```python
from build123d import *

# Parameters (mm, degrees)
EXTRUDE_1_DEPTH               = 10
EXTRUDE_2_DEPTH               = 5
EXTRUDE_2_DEPTH_BACK          = 5
EXTRUDE_2_START               = -2.5
CUT_EXTRUDE_3_DEPTH           = 308.667661103
CUT_EXTRUDE_3_DEPTH_BACK      = 308.667661103
SKETCH_4_W                    = 20
SKETCH_4_H                    = 2.700809371
CUT_EXTRUDE_2_DEPTH           = 308.667661103
CUT_EXTRUDE_2_DEPTH_BACK      = 308.667661103
SKETCH_5_W                    = 1
SKETCH_5_H                    = 14.903200109
SKETCH_8_W                    = 10
SKETCH_8_H                    = 1.5
EXTRUDE_2_2_DEPTH             = 10
EXTRUDE_2_2_DIRECTION_2_REACH = 314.682
SKETCH_11_W                   = 20
SKETCH_11_H                   = 26.003490823
CUT_EXTRUDE_4_DEPTH           = 10
EXTRUDE_3_DEPTH               = 15
CUT_EXTRUDE_5_DEPTH           = 318.837559332
CUT_EXTRUDE_5_DEPTH_BACK      = 318.837559332
SKETCH_13_R                   = 3
EXTRUDE_4_DEPTH               = 50


with BuildPart() as part:
    # 草图1 → 凸台-拉伸1 (new, symmetric)
    with BuildSketch(Plane.XY):
        Polygon((0, 0), (138.199336083, 164.699555271), (145.269999789, 173.126044145), (149.100222005, 169.912106096), (142.029558298, 161.485617222), (10.722534603, 5), (4.294658506, -2.660444431), (30, -2.660444431), (30, -7.660444431), (-6.427876097, -7.660444431), align=None)
    extrude(amount=EXTRUDE_1_DEPTH, both=True)

    # 草图3 → Extrude 2 (add, two sides: drawn at the far end of the back side and taken through both)
    with BuildSketch(Plane(origin=(0, 0, 0), x_dir=(0, 0, 1), z_dir=(-0.766044443118979, 0.642787609686538, 0)).offset(EXTRUDE_2_START - EXTRUDE_2_DEPTH_BACK)):
        with BuildLine():
            Line((-17.5, 226.389937847), (-17.5, 226.243201682))
            Line((-17.5, 226.243201682), (-17.5, 222.5))
            Line((-17.5, 222.5), (-7.5, 222.5))
            Line((-7.5, 222.5), (-7.5, 223.5))
            Line((-7.5, 223.5), (7.5, 223.5))
            Line((7.5, 223.5), (7.5, 222.5))
            Line((7.5, 222.5), (17.5, 222.5))
            Line((17.5, 222.5), (17.5, 226.243201682))
            Line((17.5, 226.243201682), (17.5, 226.389937847))
            ThreePointArc((17.5, 226.389937847), (0, 300.243201682), (-17.5, 226.389937847))
        make_face()
        with BuildLine():
            Line((-15, 227.967835418), (-15, 226.243201682))
            Line((-15, 226.243201682), (-15, 225))
            Line((-15, 225), (-10, 225))
            Line((-10, 225), (-10, 226))
            Line((-10, 226), (10, 226))
            Line((10, 226), (10, 225))
            Line((10, 225), (15, 225))
            Line((15, 225), (15, 226.243201682))
            Line((15, 226.243201682), (15, 227.967835418))
            ThreePointArc((15, 227.967835418), (0, 297.743201682), (-15, 227.967835418))
        make_face(mode=Mode.SUBTRACT)
    extrude(amount=EXTRUDE_2_DEPTH + EXTRUDE_2_DEPTH_BACK)

    # 草图4 → 切除-拉伸3 (cut, two sides: drawn at the far end of the back side and taken through both)
    with BuildSketch(Plane(origin=(0, 0, 0), x_dir=(0, 0, 1), z_dir=(-0.7660444431189785, 0.6427876096865388, 0)).offset(-CUT_EXTRUDE_3_DEPTH_BACK)):
        with Locations((0, 226.350404685)):
            Rectangle(SKETCH_4_W, SKETCH_4_H)
    extrude(amount=CUT_EXTRUDE_3_DEPTH + CUT_EXTRUDE_3_DEPTH_BACK, mode=Mode.SUBTRACT)

    # 草图5 → 切除-拉伸2 (cut, two sides: drawn at the far end of the back side and taken through both)
    with BuildSketch(Plane(origin=(0, 0, 0), x_dir=(0, 0, 1), z_dir=(-0.7660444431189785, 0.6427876096865388, 0)).offset(-CUT_EXTRUDE_2_DEPTH_BACK)):
        with Locations((0, 297.743201683)):
            Rectangle(SKETCH_5_W, SKETCH_5_H)
    extrude(amount=CUT_EXTRUDE_2_DEPTH + CUT_EXTRUDE_2_DEPTH_BACK, mode=Mode.SUBTRACT)

    # 草图8 → Extrude 2 2 (add)
    with BuildSketch(Plane(origin=(192.990549633, 229.997180861, 0), x_dir=(0.766044443118979, -0.6427876096865381, 0), z_dir=(0.6427876096865381, 0.766044443118979, 0))):
        with Locations((2.5, -1.25)):
            Rectangle(SKETCH_8_W, SKETCH_8_H)
    extrude_2_2 = extrude(amount=EXTRUDE_2_2_DEPTH)

    # 草图8 → Extrude 2 2 direction 2 (add, up to next)
    with BuildSketch(Plane(origin=(192.990549633, 229.997180861, 0), x_dir=(0.766044443118979, -0.6427876096865381, 0), z_dir=(0.6427876096865381, 0.766044443118979, 0)), mode=Mode.PRIVATE) as extrude_2_2_direction_2_sk1:
        with Locations((2.5, -1.25)):
            Rectangle(SKETCH_8_W, SKETCH_8_H)
    extrude_2_2_direction_2_tool1 = extrude(extrude_2_2_direction_2_sk1.sketch, amount=-EXTRUDE_2_2_DIRECTION_2_REACH, mode=Mode.PRIVATE) - part.part
    extrude_2_2_direction_2 = extrude_2_2_direction_2_tool1.solids().sort_by_distance((194.905661, 228.390212, 1.25))[0]
    add(extrude_2_2_direction_2)

    # 镜向1: Extrude 2 2, Extrude 2 2 direction 2 across plane
    add(extrude_2_2.mirror(Plane.XY))
    add(extrude_2_2_direction_2.mirror(Plane.XY))

    # 草图11 → 切除-拉伸4 (cut)
    with BuildSketch(Plane.XZ.offset(7.660444431)):
        with Locations((20, -3.001745411)):
            Rectangle(SKETCH_11_W, SKETCH_11_H)
    extrude(amount=-CUT_EXTRUDE_4_DEPTH, mode=Mode.SUBTRACT)

    # 草图12 → 凸台-拉伸3 (add)
    with BuildSketch(Plane.XY.offset(10)):
        Polygon((4.294658506, -2.660444431), (-2.232377941, -2.660444431), (-6.427876097, -7.660444431), (10, -7.660444431), (10, -2.660444431), align=None)
    extrude_3 = extrude(amount=EXTRUDE_3_DEPTH)

    # 镜向2: 凸台-拉伸3 across plane
    add(extrude_3.mirror(Plane.XY))

    # 草图13 → 切除-拉伸5 (cut, two sides: drawn at the far end of the back side and taken through both)
    with BuildSketch(Plane(origin=(0, 0, -2), x_dir=(-1, 0, 0), z_dir=(0, 0, -1)).offset(-CUT_EXTRUDE_5_DEPTH_BACK)):
        with Locations((-198.163787282, 232.207589437)):
            Circle(SKETCH_13_R)
    extrude(amount=CUT_EXTRUDE_5_DEPTH + CUT_EXTRUDE_5_DEPTH_BACK, mode=Mode.SUBTRACT)

    # 草图14 → 凸台-拉伸4 (add)
    with BuildSketch(Plane(origin=(0, 0, -25), x_dir=(-1, 0, 0), z_dir=(0, 0, -1))):
        Polygon((2.232377941, -2.660444431), (6.427876097, -2.660444431), (14.127876097, -2.660444431), (19.127876097, -2.660444431), (19.127876097, -7.660444431), (14.127876097, -7.660444431), (14.127876097, -14.660444431), (6.427876097, -14.660444431), (6.127876097, -14.660444431), (6.127876097, -7.660444431), (6.427876097, -7.660444431), align=None)
    extrude(amount=-EXTRUDE_4_DEPTH)


solid = part.part
```
The listing builds one solid part. Answer for the finished solid, in the listing's coordinates (mm). A direction names the side the tool comes from. Give positions to 0.01 mm unless a question says otherwise; leave off trailing zeros. Order: outer loops, then holes, each group sorted by start corner. A loop starts at its lowest first (then second) coordinate and runs counter-clockwise, first axis right, second up. Notation, with made-up numbers: (-16.75, 27.5) -> (25.25, 27.5) arc R31 cw to (25.25, 56.5) -> close; hole circle Ø3 at (28, 12). An arc over 180 degrees is marked (long way). Answer as a JSON object with one key per item and string values. Group by question number.
Item 1: The part is cut by section B-B on z = 32.5. Write down the section's boundary in (x, y).
Item 2: The part is cut by section D-D on y = 126. Write down the section's boundary in (x, z).
Item 3: Consider L1, parallel to Z at x = 146.5, y = 173; L2, parallel to Y at x = 161, z = 32; L3, parallel to Y at x = -5.5, z = 3. Determine where each line is inside the solid, lowest interval first. Write a range as from..to.
Item 4: The part is cut by section A-A on z = -31.5. Write down the section's boundary in (x, y), and give its area (3 significant figures).
Item 5: A tool of negligible diameter and unlimited length cuts with its end or side. For faces 1 (the flat face through (146, 170, 17.5)), 2 (the flat face through (195, 231, 0.5)), 3 (the cylindrical face through (174.23, 203.64, 35.87)), from which of +Z, -Z, +X, -X, +Y, -Y can it reach the whole face along a straight path? Write none if from no direction.
Item 6: Determine the mould class of faces 4 (the flat face through (149.942, 167.025, -0.182)), 5 (the flat face through (146.596, 170.708, -0.21)), 6 (the cylindrical face through (175.495, 205.149, -38.014)) for opening direction Z: pulls with the +Z half, pulls with the -Z half, needs draft (parallel to the pull), parting line crosses it, or undercut.
Item 7: Flat-ended cylindrical pins translate along their axes: pin 1 (2.5 mm diameter, centred on y = -6.5, z = 9, fed in from +X); pin 2 (4.5 mm diameter, centred on x = 146, y = 174, fed in from +Z); pin 3 (6 mm diameter, centred on x = -10.5, y = -9.5, fed in from +Z); pin 4 (12 mm diameter, centred on x = 88.5, y = 83, fed in from -Z). Find the tip coordinate at first contact, or state that the pin passes through.
Item 8: The part is cut by section C-C on x = 50. Write down the section's boundary in (y, z), and give its area (3 significant figures).
Result set:
{
 "1": {"outline": "(152.15, 185.22) -> (159.81, 178.79) -> (162.99, 182.58) -> (155.33, 189) -> close; (176.69, 214.46) -> (184.35, 208.03) -> (187.53, 211.82) -> (179.87, 218.25) -> close"},
 "2": {"outline": "(105.73, -10) -> (112.25, -10) -> (112.25, 10) -> (105.73, 10) -> close"},
 "3": {"L1": "-18.09..-15, 15..18.09", "L2": "180.2..183.01", "L3": "-7.66..-2.66"},
 "4": {"outline": "(151.23, 184.12) -> (158.89, 177.69) -> (161.82, 181.18) -> (154.16, 187.61) -> close; (177.86, 215.86) -> (185.52, 209.43) -> (188.45, 212.92) -> (180.79, 219.35) -> close", "area": "91.1 mm²"},
 "5": {"face 1": "+Z, -X, -Y", "face 2": "+X, -X, +Y, -Y", "face 3": "none"},
 "6": {"face 4": "needs draft", "face 5": "undercut", "face 6": "pulls with the -Z half"},
 "7": {"pin 1": "x = 10", "pin 2": "z = 22.5", "pin 3": "z = 25", "pin 4": "through"},
 "8": {"outline": "(51.81, -10) -> (59.59, -10) -> (59.59, 10) -> (51.81, 10) -> close", "area": "156 mm²"}
}
